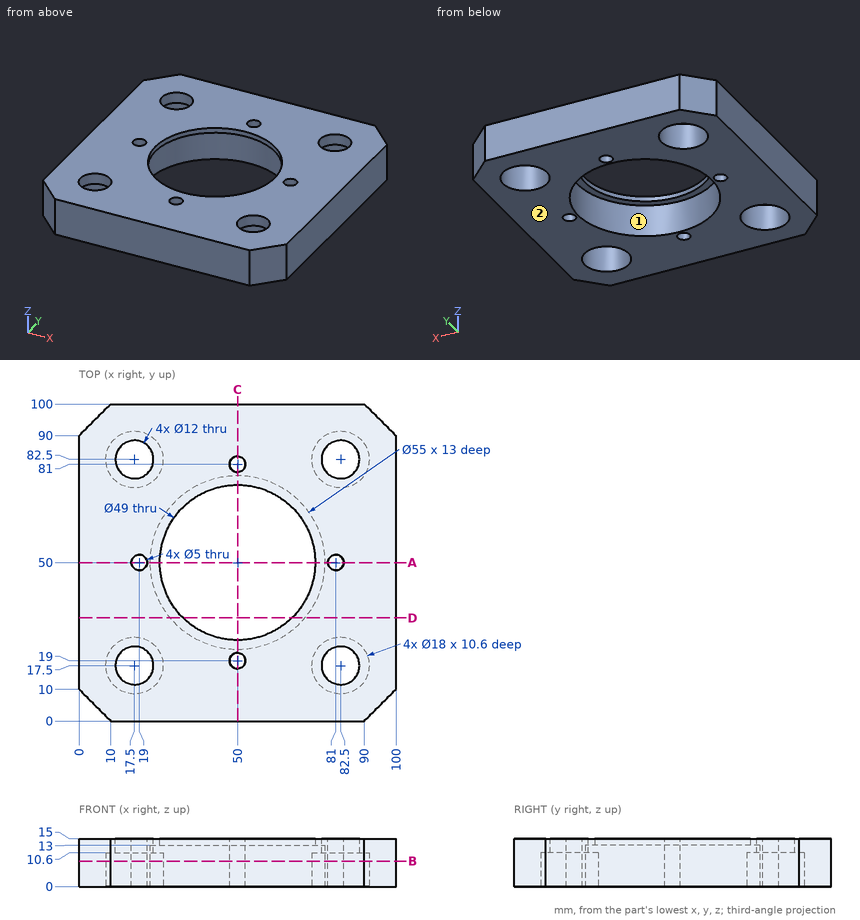
Can you work these out from the drawing? Everything is in mm from the part's minimum corner. A direction names the side the tool comes from. Round coordinates to 2 decimals unless told otherwise and drop trailing zeros. Loops run counter-clockwise (first coordinate to the right, second up) from the corner with the lowest first, then second, coordinate; pieces in that order, holes last. Notation, with made-up numbers: (17, 13.25) -> (70, 13.25) arc R10 ccw to (70, 19.25) -> close; hole circle Ø2 at (-26.5, -21.5). An arc over 180 degrees is marked (long way). Use CSV: the item, a comma, the result in double quotes.
(1) If I drill on probe 1 along Y at (x, z) = (50, 5.5); probe 2 along Y at (x, z) = (17, 9.5); probe 3 along X at (y, z) = (48.5, 5), over which ranges is the centre line in solid material (lowest first)? Write a range as [from, to].
Return value:
probe 1,"y = [0, 16.5], [21.5, 22.5], [77.5, 78.5], [83.5, 100]"
probe 2,"y = [0, 8.51], [26.49, 48.5], [51.5, 73.51], [91.49, 100]"
probe 3,"x = [0, 17], [21, 22.54], [77.46, 79], [83, 100]"
(2) Suppose I cut it at D-D on y = 32.5. Write out the boundary of the cut face in (x, z), plus the area to 3 significant figures.
Return value:
outline,"(0, 0) -> (28.79, 0) -> (28.79, 13) -> (32.85, 13) -> (32.85, 15) -> (0, 15) -> close; (67.15, 13) -> (71.21, 13) -> (71.21, 0) -> (100, 0) -> (100, 15) -> (67.15, 15) -> close"
area,"880 mm²"
(3) Suppose I cut it at B-B on z = 8. Give the number of separate pieces and of enclosed holes in the cut face, plus the area to 3 significant figures.
Return value:
separate pieces,"1"
enclosed holes,"9"
area,"6,330 mm²"
(4) Suppose I cut it at A-A on y = 50. Write out the boundary of the cut face in (x, z), plus the area to 3 significant figures.
Return value:
outline,"(0, 0) -> (16.5, 0) -> (16.5, 15) -> (0, 15) -> close; (21.5, 0) -> (22.5, 0) -> (22.5, 13) -> (25.5, 13) -> (25.5, 15) -> (21.5, 15) -> close; (74.5, 13) -> (77.5, 13) -> (77.5, 0) -> (78.5, 0) -> (78.5, 15) -> (74.5, 15) -> close; (83.5, 0) -> (100, 0) -> (100, 15) -> (83.5, 15) -> close"
area,"537 mm²"
(5) For the marked faces 1 and 2, which set-ups out of +Z, -Z, +X, -X, +Y, -Y let a thin tool reach every point of the face, with its end or its side?
Return value:
face 1,"-Z"
face 2,"-Z, +X, -X, +Y, -Y"
(6) Will these pins go through, and if not, where does the flat tip stop? pin 1 Ø7 at (x, y) = (82.5, 17.5) entering from +Z; pin 2 Ø5.5 at (x, y) = (15.5, 86) entering from -Z.
Return value:
pin 1,"passes through"
pin 2,"stops at z = 10.6"
